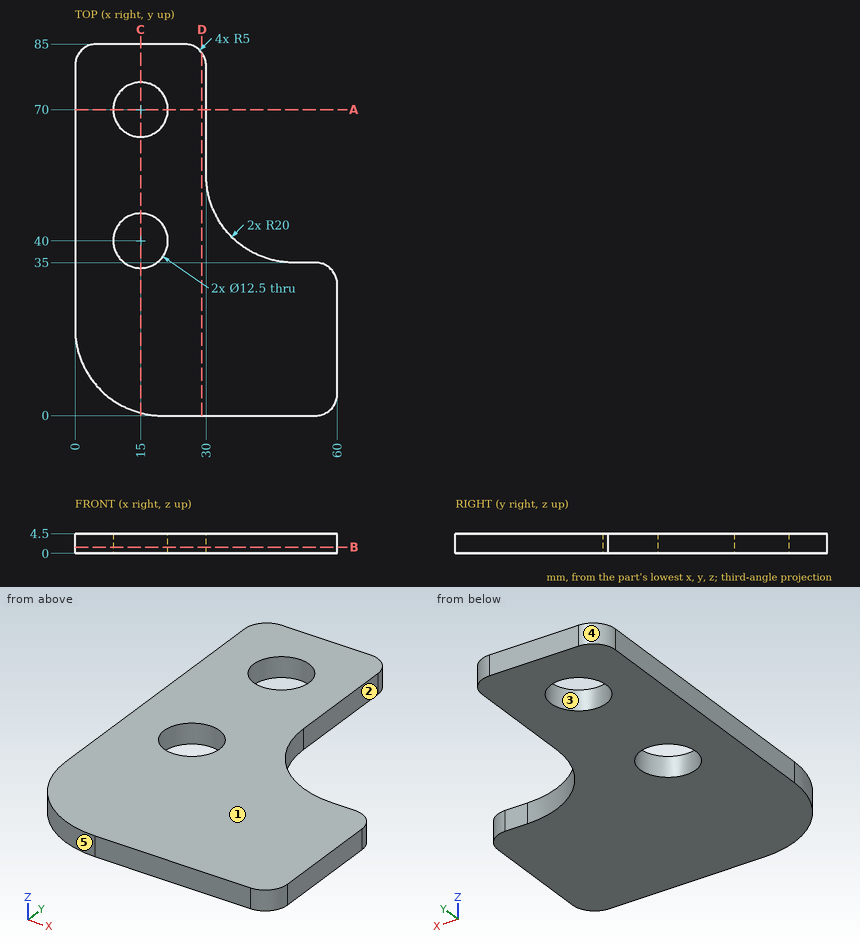
Geometry check sheet. Reference: drawing and pictorial views, mm from the part's lowest x, y, z. A direction names the side the tool comes from. Give positions to 0.01 mm unless a question says otherwise; leave off trailing zeros. Order: outer loops, then holes, each group sorted by start corner. A loop starts at its lowest first (then second) coordinate and runs counter-clockwise, first axis right, second up. Notation, with made-up numbers: M -19.5,72 L 16.5,72 A32 cw 16.5,104 Z; hole C 80,-12.75 d11. An arc over 180 degrees is marked long. Answer in a Markdown table with one row per item. Add a question column.
Q1. Sectioned sample at C-C, the plane x = 15. Record the boundary of the cut face in (y, z).
Q2. Gauge pin test, flat ends, axial feed: pin 1 Ø2 at (y, z) = (72, 1.5) entering from +X; pin 2 Ø7.5 at (x, y) = (15, 40) entering from -Z. Record the tip position at first contact, or that the pin passes through.
Q3. Thickness scan on L1, parallel to Y at x = 15, z = 3.05; L2, parallel to X at y = 69, z = 1.2; L3, parallel to X at y = 40.5, z = 2.6. Record the ranges inside material, lowest first.
Q4. Access from +Z, -Z, +X, -X, +Y, -Y to the whole of each face (thin tool, end or side, straight path). Record for the marked faces 1 and 2.
Q5. Sectioned sample at A-A, the plane y = 70. Record the boundary of the cut face in (x, z), and give its area (4 significant figures).
Q6. Sectioned sample at D-D, the plane x = 29. Record the boundary of the cut face in (y, z).
Q7. Release check for a two-part mould opening along Y. For the marked faces 3, 4 and 5 record: released by +Y, released by -Y, zero draft, split by the parting line, or undercut.
Q8. Sectioned sample at B-B, the plane z = 1.4. Record the boundary of the cut face in (x, y), and give its area (3 significant figures).
Verdict:
| question | item | result |
|---|---|---|
| 1 | outline | M 0.64,0 L 33.75,0 L 33.75,4.5 L 0.64,4.5 Z; M 46.25,0 L 63.75,0 L 63.75,4.5 L 46.25,4.5 Z; M 76.25,0 L 85,0 L 85,4.5 L 76.25,4.5 Z |
| 2 | pin 1 | x = 30 |
| 2 | pin 2 | through |
| 3 | L1 | 0.64 to 33.75, 46.25 to 63.75, 76.25 to 85 |
| 3 | L2 | 0 to 8.83, 21.17 to 30 |
| 3 | L3 | 0 to 8.77, 21.23 to 36.23 |
| 4 | face 1 | +Z, +X, -X, +Y, -Y |
| 4 | face 2 | +Z, -Z, +X, +Y |
| 5 | outline | M 0,0 L 8.75,0 L 8.75,4.5 L 0,4.5 Z; M 21.25,0 L 30,0 L 30,4.5 L 21.25,4.5 Z |
| 5 | area | 78.75 mm² |
| 6 | outline | M 0,0 L 83,0 L 83,4.5 L 0,4.5 Z |
| 7 | face 3 | undercut |
| 7 | face 4 | released by +Y |
| 7 | face 5 | released by -Y |
| 8 | outline | M 0,20 A20 ccw 20,0 L 55,0 A5 ccw 60,5 L 60,30 A5 ccw 55,35 L 50,35 A20 cw 30,55 L 30,80 A5 ccw 25,85 L 5,85 A5 ccw 0,80 Z; hole C 15,40 d12.5; hole C 15,70 d12.5 |
| 8 | area | 3,330 mm² |
